```python
from build123d import *

# Parameters (mm, degrees)
SKETCH2_R          = 3.5
CUT_EXTRUDE1_DEPTH = 118.798556867
CIRPATTERN1_COUNT  = 4


with BuildPart() as part:
    # Sketch1 → Revolve1 (revolve)
    with BuildSketch(Plane.XY):
        Polygon((-50, 0), (-72.5, 0), (-72.5, 2), (-52, 2), (-52, 60), (0, 60), (0, 58), (-50, 58), align=None)
    revolve(axis=Axis((0, 60, 0), (0, -1, 0)))

    # Sketch2 → Cut-Extrude1 (cut, through all)
    with BuildSketch(Plane(origin=(0, 2, 0), x_dir=(1, 0, 0), z_dir=(0, 1, 0))):
        with Locations(Location((0, 62.5, 0), (0, 0, 180))):
            Circle(SKETCH2_R)
    cut_extrude1 = extrude(amount=-CUT_EXTRUDE1_DEPTH, mode=Mode.SUBTRACT)

    # CirPattern1: Cut-Extrude1 ×4 about axis
    cirpattern1_axis = Axis((0, 0, 0), (0, 1, 0))
    for i in range(1, CIRPATTERN1_COUNT):
        add(cut_extrude1.rotate(cirpattern1_axis, i * 360 / CIRPATTERN1_COUNT), mode=Mode.SUBTRACT)


solid = part.part
```
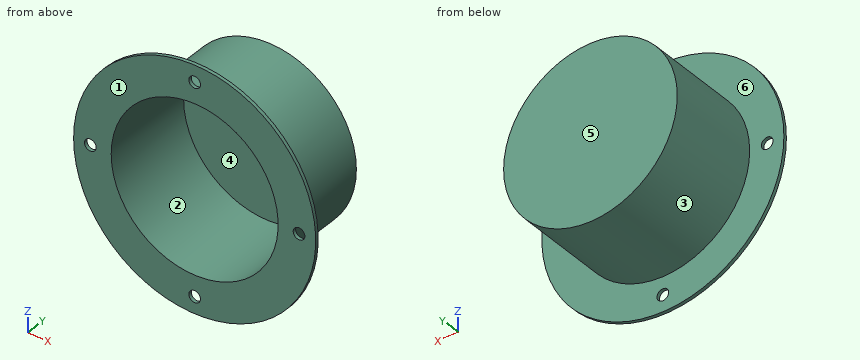
For this review, take the finished solid that the model builds, in its own axes (mm). Face numbers are marked on the shaded views. A direction names the side the tool comes from. Coordinates: 2 decimals unless noted, no trailing zeros. Order: outer loops, then holes, each group sorted by start corner. A loop starts at its lowest first (then second) coordinate and runs counter-clockwise, first axis right, second up. Notation, with made-up numbers: (53, 16.5) - (78, 16.5) arc R23 ccw to (78, 47.5) - close; hole circle Ø7 at (-20.5, 80). An arc over 180 degrees is marked (long way). Answer as a JSON object with one key per item and string values. Group by question number.
1. We need section B-B on z = 0. State the section outline as (x, y) points, then the cut area to 3 significant figures.
2. Clearance check with flat-ended pins moving along their axes: P1, Ø1, axis at x = 55.5, z = -34, coming from the -Y side; P2, Ø3, axis at y = 16, z = -22.5, coming from the -X side; P3, Ø3, axis at y = 16, z = -45, coming from the -X side; P4, Ø6, axis at x = -53.5, z = -24.5, coming from the +Y side. State where each tip first meets the part, or that it passes through.
3. The part is to be moulded in two halves that separate along Z. For the marked faces 1, 2 and 3, say which applies: pulls with the +Z half, pulls with the -Z half, needs draft (parallel to the pull), parting line crosses it, or undercut.
4. For probe 1 along Z at (x, y) = (0, 1.5); probe 2 along X at (y, z) = (43.5, 0), list the stretches that pass through material, from the lowest coordinate up.
5. For the marked faces 4, 5 and 6, list the 3-axis set-ups (+Z, -Z, +X, -X, +Y, -Y) from which the entire face can be reached by the end or side of a thin tool; tool diameter is ignored.
6. We need section D-D on z = 62.5. State the section outline as (x, y) points.
7. We need section A-A on x = 0. State the section outline as (y, z) points, then the cut area to 3 significant figures.
8. We need section C-C on x = -62.5. State the section outline as (y, z) points, then the cut area to 3 significant figures.
Final values:
{
 "1": {"outline": "(-72.5, 0) - (-66, 0) - (-66, 2) - (-72.5, 2) - close; (-59, 0) - (-50, 0) - (-50, 58) - (50, 58) - (50, 0) - (59, 0) - (59, 2) - (52, 2) - (52, 60) - (-52, 60) - (-52, 2) - (-59, 2) - close; (66, 0) - (72.5, 0) - (72.5, 2) - (66, 2) - close", "area": "494 mm²"},
 "2": {"P1": "y = 0", "P2": "x = -47.57", "P3": "x = -28.49", "P4": "y = 2"},
 "3": {"face 1": "needs draft", "face 2": "undercut", "face 3": "parting line crosses it"},
 "4": {"probe 1": "-72.5 to -66, -59 to -50, 50 to 59, 66 to 72.5", "probe 2": "-52 to -50, 50 to 52"},
 "5": {"face 4": "-Y", "face 5": "+Z, -Z, +X, -X, +Y", "face 6": "+Y"},
 "6": {"outline": "(-36.74, 0) - (-3.5, 0) - (-3.5, 2) - (-36.74, 2) - close; (3.5, 0) - (36.74, 0) - (36.74, 2) - (3.5, 2) - close"},
 "7": {"outline": "(0, -72.5) - (2, -72.5) - (2, -66) - (0, -66) - close; (0, -59) - (2, -59) - (2, -52) - (60, -52) - (60, 52) - (2, 52) - (2, 59) - (0, 59) - (0, 50) - (58, 50) - (58, -50) - (0, -50) - close; (0, 66) - (2, 66) - (2, 72.5) - (0, 72.5) - close", "area": "494 mm²"},
 "8": {"outline": "(0, -36.74) - (2, -36.74) - (2, -3.5) - (0, -3.5) - close; (0, 3.5) - (2, 3.5) - (2, 36.74) - (0, 36.74) - close", "area": "133 mm²"}
}
